Verification items for the finished model (mm, model axes). Face numbers are marked on the shaded views. A direction names the side the tool comes from. Coordinates: 2 decimals unless noted, no trailing zeros. Write each loop counter-clockwise with the first axis right and the second up, starting at its lowest first coordinate (ties: lowest second). Pieces come first, ordered by that corner, then holes. Notation, with made-up numbers: (20, 72.25) - (33, 72.25) arc R12 cw to (33, 90.25) - close; hole circle Ø10 at (57, -1). An arc over 180 degrees is marked (long way). Use one line per item in the form item = value. Start each with the question number.
(1) Mould release check, pull along X, two halves, no side actions. Record for the marked faces 4, 5 and 6: released by +X, released by -X, zero draft, split by the parting line, or undercut.
(2) Gauge pin test, flat ends, axial feed: pin 1 Ø10 at (x, y) = (-3.5, 59.5) entering from -Z; pin 2 Ø1.5 at (y, z) = (91.5, -19.5) entering from -X; pin 3 Ø12 at (x, y) = (6.5, 52.5) entering from +Z; pin 4 Ø21.5 at (x, z) = (0, 0) entering from +Y. Record the tip position at first contact, or that the pin passes through.
(3) Tool access check on the marked faces 1, 2 and 3. Record the directions out of +Z, -Z, +X, -X, +Y, -Y that give a thin tool (end or side, any length) a straight path to the whole face; none if there is none.
(4) Sectioned sample at A-A (z = 0). Record the cut outline in (x, y).
(5) Material ranges on line 1 (X direction, y = 8, z = 0); line 2 (Y direction, x = -4, z = 12); line 3 (Y direction, x = 27, z = 10.5), recorded low to high. Write a range as [from, to].
(6) Sectioned sample at C-C (y = 9). Record the cut outline in (x, z).
(7) Sectioned sample at B-B (x = 0). Record the cut outline in (y, z), and give its area (3 significant figures).
(8) Sectioned sample at D-D (y = 55). Record the cut outline in (x, z).
from build123d import *

# Parameters (mm, degrees)
SKETCH_2_R          = 12
CUT_EXTRUDE_1_DEPTH = 116.5
SKETCH_3_R          = 23.5
SKETCH_3_R_2        = 10
CUT_EXTRUDE_2_DEPTH = 17
CUT_EXTRUDE_START   = -17
SKETCH_4_R          = 23.5
SKETCH_4_R_2        = 10
CUT_EXTRUDE_3_DEPTH = 17
FILLET_1_R          = 1


with BuildPart() as part:
    # 草图1 → 旋转1 (revolve)
    with BuildSketch(Plane.XY, mode=Mode.PRIVATE) as revolve_1_sk:
        with BuildLine():
            Line((0, 0), (0, 116.5))
            Line((0, 116.5), (30, 116.5))
            Line((30, 116.5), (30, 101.5))
            ThreePointArc((30, 101.5), (20, 58.25), (30, 15))
            Line((30, 15), (30, 0))
            Line((30, 0), (0, 0))
        make_face()
    revolve(revolve_1_sk.sketch.rotate(Axis((0, 0, 0), (0, 1, 0)), 90), axis=Axis((0, 0, 0), (0, 1, 0)))

    # 草图2 → 切除-拉伸1 (cut)
    with BuildSketch(Plane(origin=(0, 116.5, 0), x_dir=(1, 0, 0), z_dir=(0, 1, 0))):
        with Locations(Location((0, 0, 0), (0, 0, 270))):
            Circle(SKETCH_2_R)
    extrude(amount=-CUT_EXTRUDE_1_DEPTH, mode=Mode.SUBTRACT)

    # 草图3 → 切除-拉伸2 (cut)
    with BuildSketch(Plane(origin=(0, 116.5, 0), x_dir=(1, 0, 0), z_dir=(0, 1, 0))):
        with Locations(Location((0, 0, 0), (0, 0, 270))):
            Circle(SKETCH_3_R)
        Circle(SKETCH_3_R_2, mode=Mode.SUBTRACT)
    extrude(amount=-CUT_EXTRUDE_2_DEPTH, mode=Mode.SUBTRACT)

    # 草图4 → 切除-拉伸3 (cut)
    with BuildSketch(Plane.XZ.offset(CUT_EXTRUDE_START)):
        with Locations(Location((0, 0, 0), (0, 0, 90))):
            Circle(SKETCH_4_R)
        Circle(SKETCH_4_R_2, mode=Mode.SUBTRACT)
    extrude(amount=CUT_EXTRUDE_3_DEPTH, mode=Mode.SUBTRACT)

    # 圆角1
    fillet_1_edges = [part.edges().sort_by_distance(p)[0] for p in [
        (0, 116.5, 30),
        (0, 0, 30),
    ]]
    fillet(fillet_1_edges, radius=FILLET_1_R)


solid = part.part
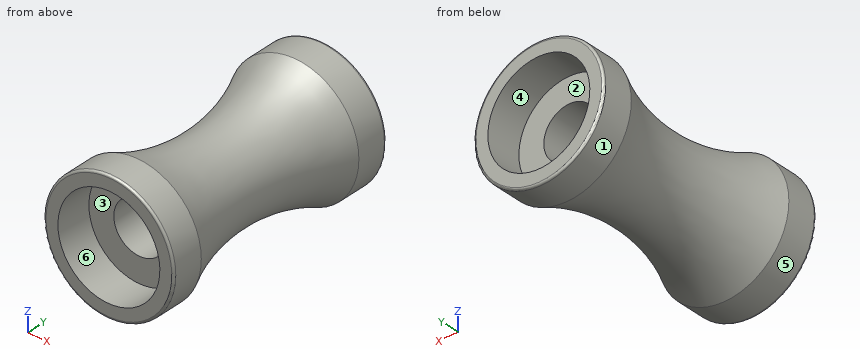
Answers below:
q1.face_4 = undercut
q1.face_5 = split by the parting line
q1.face_6 = undercut
q2.pin_1 = -20.14
q2.pin_2 = -17.79
q2.pin_3 = 20.38
q2.pin_4 = through
q3.face_1 = +Y, -Y
q3.face_2 = +Y
q3.face_3 = -Y
q4.outline = (-30, 1) arc R1 ccw to (-29, 0) - (-23.5, 0) - (-23.5, 17) - (-12, 17) - (-12, 99.5) - (-23.5, 99.5) - (-23.5, 116.5) - (-29, 116.5) arc R1 ccw to (-30, 115.5) - (-30, 101.5) arc R98.53 cw to (-30, 15) - close; (12, 17) - (23.5, 17) - (23.5, 0) - (29, 0) arc R1 ccw to (30, 1) - (30, 15) arc R98.53 cw to (30, 101.5) - (30, 115.5) arc R1 ccw to (29, 116.5) - (23.5, 116.5) - (23.5, 99.5) - (12, 99.5) - close
q5.line_1 = [-30, -23.5], [23.5, 30]
q5.line_2 = [17, 99.5]
q5.line_3 = [0, 17.18], [99.32, 116.5]
q6.outline = circle Ø60 at (0, 0); hole circle Ø47 at (0, 0)
q7.outline = (0, -29) arc R1 ccw to (1, -30) - (15, -30) arc R98.53 cw to (101.5, -30) - (115.5, -30) arc R1 ccw to (116.5, -29) - (116.5, -23.5) - (99.5, -23.5) - (99.5, -12) - (17, -12) - (17, -23.5) - (0, -23.5) - close; (0, 23.5) - (17, 23.5) - (17, 12) - (99.5, 12) - (99.5, 23.5) - (116.5, 23.5) - (116.5, 29) arc R1 ccw to (115.5, 30) - (101.5, 30) arc R98.53 cw to (15, 30) - (1, 30) arc R1 ccw to (0, 29) - close
q7.area = 2,250 mm2
q8.outline = circle Ø40.11 at (0, 0); hole circle Ø24 at (0, 0)
